Design review of the part built by this model. Coordinates are the model's own, in mm. Coordinates: 2 decimals unless noted, no trailing zeros. Write each loop counter-clockwise with the first axis right and the second up, starting at its lowest first coordinate (ties: lowest second). Pieces come first, ordered by that corner, then holes.
Q1. Take a section at A-A, the plane x = 0. Write out the cut boundary in (y, z), plus the area to 3 significant figures.
Q2. For L1, parallel to Y at x = 0, z = 8.25; L2, parallel to Y at x = 6, z = 4.25; L3, parallel to X at y = -1, z = 2.75, list the stretches that pass through material, from the lowest coordinate up.
Q3. Take a section at C-C, the plane z = 8. Write out the cut boundary in (x, y), plus the area to 3 significant figures.
Q4. Take a section at B-B, the plane y = 8.5. Write out the cut boundary in (x, z), plus the area to 3 significant figures.
Q5. For pin 1 Ø3 at (x, z) = (-18, 4.5) entering from -Y; pin 2 Ø3 at (y, z) = (-4.5, 5.5) entering from +X, all flat-tipped, find the tip position at first contact; note any pin that passes through.
Q6. The part is to be moulded in two halves that separate along X. For faces 1 (the cylindrical face through (-3.27, -14.74, 4.93)), 2 (the flat face through (30, 52, 5)), 3 (the flat face through (-30, 52, 5)), 4 (the flat face through (0, -20, 5)), say which applies: released by +X, released by -X, zero draft, split by the parting line, or undercut.
from build123d import *

# Parameters (mm, degrees)
SKETCH_1_W      = 60
SKETCH_1_H      = 125
SKETCH_1_R      = 15.1
EXTRUDE_1_DEPTH = 10
FILLET_1_R      = 20


with BuildPart() as part:
    # 草图1 → 凸台-拉伸1 (new body)
    with BuildSketch(Plane.XY):
        with Locations((0, 42.5)):
            Rectangle(SKETCH_1_W, SKETCH_1_H)
        Circle(SKETCH_1_R, mode=Mode.SUBTRACT)
    extrude(amount=EXTRUDE_1_DEPTH)

    # 圆角1
    fillet_1_edges = [part.edges().sort_by_distance(p)[0] for p in [
        (30, -20, 5),
        (-30, -20, 5),
    ]]
    fillet(fillet_1_edges, radius=FILLET_1_R)


solid = part.part
Responses:
1. outline: (-20, 0) - (-15.1, 0) - (-15.1, 10) - (-20, 10) - close; (15.1, 0) - (105, 0) - (105, 10) - (15.1, 10) - close
1. area: 948 mm2
2. L1: y = -20 to -15.1, 15.1 to 105
2. L2: y = -20 to -13.86, 13.86 to 105
2. L3: x = -29.97 to -15.07, 15.07 to 29.97
3. outline: (-30, 0) arc R20 ccw to (-10, -20) - (10, -20) arc R20 ccw to (30, 0) - (30, 105) - (-30, 105) - close; hole circle Ø30.2 at (0, 0)
3. area: 6,610 mm2
4. outline: (-30, 0) - (-12.48, 0) - (-12.48, 10) - (-30, 10) - close; (12.48, 0) - (30, 0) - (30, 10) - (12.48, 10) - close
4. area: 350 mm2
5. pin 1: stops at y = -18.91
5. pin 2: stops at x = 29.77
6. face 1: undercut
6. face 2: released by +X
6. face 3: released by -X
6. face 4: zero draft
